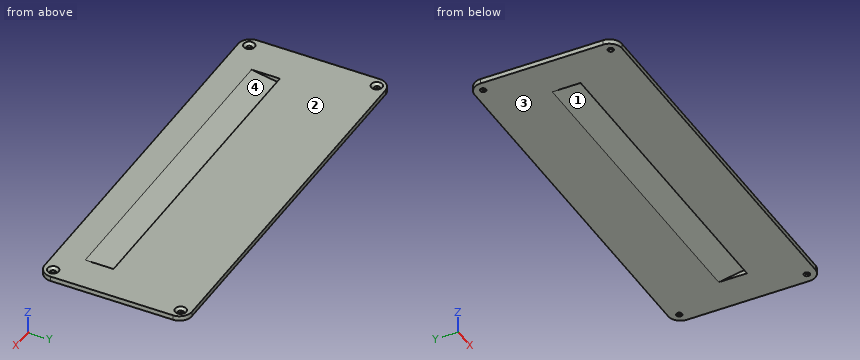
```python
from build123d import *

# Parameters (mm, degrees)
SKETCH1_W                                         = 160
SKETCH1_H                                         = 60
BOSS_EXTRUDE1_DEPTH                               = 2
SKETCH2_R                                         = 0.5
CUT_EXTRUDE1_DEPTH                                = 2
PILOT_HOLE_SIZE_PER_CROSS_SLOTTED_COU_D           = 2.4
PILOT_HOLE_SIZE_PER_CROSS_SLOTTED_COU_DEPTH       = 7.5
PILOT_HOLE_SIZE_PER_CROSS_SLOTTED_COU_CSINK_D     = 4.5
PILOT_HOLE_SIZE_PER_CROSS_SLOTTED_COU_CSINK_ANGLE = 90
PILOT_HOLE_SIZE_PER_CROSS_SLOTTED_COU_TIP         = 0.721032743
SKETCH6_W                                         = 128.916628893
SKETCH6_H                                         = 2
CUT_EXTRUDE3_DEPTH                                = 100
FILLET1_R                                         = 5


with BuildPart() as part:
    # Sketch1 → Boss-Extrude1 (new body)
    with BuildSketch(Plane.XY):
        Rectangle(SKETCH1_W, SKETCH1_H)
    extrude(amount=BOSS_EXTRUDE1_DEPTH)

    # Sketch2 → Cut-Extrude1 (cut)
    with BuildSketch(Plane.XY.offset(2)):
        with Locations((-76, 26)):
            Circle(SKETCH2_R)
        with Locations(Location((76, 26, 0), (0, 0, 180))):
            Circle(SKETCH2_R)
        with Locations((76, -26)):
            Circle(SKETCH2_R)
        with Locations(Location((-76, -26, 0), (0, 0, 180))):
            Circle(SKETCH2_R)
    extrude(amount=-CUT_EXTRUDE1_DEPTH, mode=Mode.SUBTRACT)

    # Pilot hole size (% per cross) slotted countersunk wood screw type1
    with Locations(Plane.XY.offset(2)):
        with Locations((-76, 26), (76, 26), (76, -26), (-76, -26)):
            CounterSinkHole(PILOT_HOLE_SIZE_PER_CROSS_SLOTTED_COU_D / 2, PILOT_HOLE_SIZE_PER_CROSS_SLOTTED_COU_CSINK_D / 2, depth=PILOT_HOLE_SIZE_PER_CROSS_SLOTTED_COU_DEPTH, counter_sink_angle=PILOT_HOLE_SIZE_PER_CROSS_SLOTTED_COU_CSINK_ANGLE)
            with Locations((0, 0, -(PILOT_HOLE_SIZE_PER_CROSS_SLOTTED_COU_DEPTH + PILOT_HOLE_SIZE_PER_CROSS_SLOTTED_COU_TIP / 2))):  # 118° drill point
                Cone(0, PILOT_HOLE_SIZE_PER_CROSS_SLOTTED_COU_D / 2, PILOT_HOLE_SIZE_PER_CROSS_SLOTTED_COU_TIP, mode=Mode.SUBTRACT)

    # Sketch6 → Cut-Extrude3 (cut)
    with BuildSketch(Plane(origin=(0, -29.437409455, 5.190609529), x_dir=(1, 0, 0), z_dir=(0, -0.9848077530122086, 0.17364817766692736))):
        with Locations((0.971111813, -0.2388368)):
            Rectangle(SKETCH6_W, SKETCH6_H)
    extrude(amount=-CUT_EXTRUDE3_DEPTH, mode=Mode.SUBTRACT)

    # Fillet1
    fillet1_edges = [part.edges().sort_by_distance(p)[0] for p in [
        (80, -30, 1),
        (-80, -30, 1),
        (-80, 30, 1),
        (80, 30, 1),
    ]]
    fillet(fillet1_edges, radius=FILLET1_R)


solid = part.part
```
Here's how the part is built. I have some questions about the finished solid (model axes, mm). Face numbers are marked on the shaded views. A direction names the side the tool comes from. Coordinates: 2 decimals unless noted, no trailing zeros. Write each loop counter-clockwise with the first axis right and the second up, starting at its lowest first coordinate (ties: lowest second). Pieces come first, ordered by that corner, then holes. Notation, with made-up numbers: (33.5, 26.25) -> (87.5, 26.25) arc R16 cw to (87.5, 57.25) -> close; hole circle Ø2 at (-34.75, 36). An arc over 180 degrees is marked (long way). Use a Markdown table: item, result. Add a question column.
(1) Please list where these lines run through material, in increasing order: line 1 (Y direction, x = -76, z = 0.7); line 2 (X direction, y = 26, z = 0.7); line 3 (X direction, y = -25.5, z = 1.35).
(2) If we section it at A-A, the plane x = 59: Write out the boundary of the cut face in (y, z), and give its area (3 significant figures).
(3) We'd pull the mould along X, two halves only. Please class the marked faces 1 and 2: +X half, -X half, draft (parallel to the pull), parting line (faces both ways), or undercut.
(4) I'm going to push flat-ended pins straight in: P1, Ø1.9, axis at x = -76, y = 26, coming from the +Z side; P2, Ø1, axis at x = 15.5, y = 0, coming from the -Z side; P3, Ø6, axis at x = 9, y = -10.5, coming from the +Z side. Where does each tip first touch, or does it pass through?
(5) For the marked faces 3 and 4, which set-ups out of +Z, -Z, +X, -X, +Y, -Y let a thin tool reach every point of the face, with its end or its side?
(6) If we section it at B-B, the plane z = 1.3: Write out the boundary of the cut face in (x, y).
Outcome:
| question | item | result |
|---|---|---|
| 1 | line 1 | y = -29.9 to -27.2, -24.8 to 24.8, 27.2 to 29.9 |
| 1 | line 2 | x = -79.9 to -77.2, -74.8 to 74.8, 77.2 to 79.9 |
| 1 | line 3 | x = -79.97 to -77.52, -74.48 to 74.48, 77.52 to 79.97 |
| 2 | outline | (-30, 0) -> (-7.13, 0) -> (-18.48, 2) -> (-30, 2) -> close; (-6.96, 2) -> (4.38, 0) -> (30, 0) -> (30, 2) -> close |
| 2 | area | 97.0 mm^2 |
| 3 | face 1 | undercut |
| 3 | face 2 | draft |
| 4 | P1 | passes through |
| 4 | P2 | stops at z = 0.68 |
| 4 | P3 | stops at z = 1.12 |
| 5 | face 3 | -Z, +X, -X, +Y, -Y |
| 5 | face 4 | +Z |
| 6 | outline | (-80, -25) arc R5 ccw to (-75, -30) -> (75, -30) arc R5 ccw to (80, -25) -> (80, 25) arc R5 ccw to (75, 30) -> (-75, 30) arc R5 ccw to (-80, 25) -> close; hole circle Ø3.1 at (-76, -26); hole circle Ø3.1 at (-76, 26); hole (-63.49, -14.51) -> (65.43, -14.51) -> (65.43, -2.99) -> (-63.49, -2.99) -> close; hole circle Ø3.1 at (76, -26); hole circle Ø3.1 at (76, 26) |
